```python
from build123d import *

# Parameters (mm, degrees)
EXTRUDE_THIN1_DEPTH  = 100
SKETCH2_R            = 5
CUT_EXTRUDE1_DEPTH   = 10
LPATTERN1_COUNT      = 2
LPATTERN1_PITCH      = 70
SKETCH3_R            = 5
CUT_EXTRUDE2_DEPTH   = 10
LPATTERN2_COUNT      = 3
LPATTERN2_PITCH      = 260
LPATTERN2_COUNT_DIR2 = 2
LPATTERN2_PITCH_DIR2 = 70
SKETCH4_R            = 5
CUT_EXTRUDE3_DEPTH   = 10
LPATTERN3_COUNT      = 2
LPATTERN3_PITCH      = 70


with BuildPart() as part:
    # Sketch1 → Extrude-Thin1 (new body)
    with BuildSketch(Plane.XY):
        with BuildLine():
            Line((0, 0), (0, 126.921326068))
            ThreePointArc((0, 126.921326068), (6.221950993, 145.213520727), (22.306959029, 155.918172804))
            Line((22.306959029, 155.918172804), (735, 345))
            Line((735, 345), (736.282173495, 340.167192211))
            Line((736.282173495, 340.167192211), (23.589132524, 151.085365014))
            ThreePointArc((23.589132524, 151.085365014), (10.184959161, 142.164821617), (5, 126.921326068))
            Line((5, 126.921326068), (5, 0))
            Line((5, 0), (0, 0))
        make_face()
    extrude(amount=EXTRUDE_THIN1_DEPTH)

    # Sketch2 → Cut-Extrude1 (cut)
    with BuildSketch(Plane(origin=(-37.178988327, 140.13618677, 0), x_dir=(0.9665615578617778, 0.25643469902455335, 0), z_dir=(-0.25643469902455335, 0.9665615578617778, 0))):
        with Locations(Location((686.892716192, -15, 0), (0, 0, 180))):
            Circle(SKETCH2_R)
    cut_extrude1 = extrude(amount=-CUT_EXTRUDE1_DEPTH, mode=Mode.SUBTRACT)

    # LPattern1: Cut-Extrude1 ×2
    with Locations(*[(0, 0, i * LPATTERN1_PITCH) for i in range(1, LPATTERN1_COUNT)]):
        add(cut_extrude1, mode=Mode.SUBTRACT)

    # Sketch3 → Cut-Extrude2 (cut)
    with BuildSketch(Plane(origin=(-37.178988327, 140.13618677, 0), x_dir=(0.9665615578617778, 0.25643469902455335, 0), z_dir=(-0.25643469902455335, 0.9665615578617778, 0))):
        with Locations(Location((612.892716192, -15, 0), (0, 0, 180))):
            Circle(SKETCH3_R)
    cut_extrude2 = extrude(amount=-CUT_EXTRUDE2_DEPTH, mode=Mode.SUBTRACT)

    # LPattern2: Cut-Extrude2 3 × 2
    with Locations(*[Vector(-0.9665615578617778, -0.25643469902455335, 0) * (i * LPATTERN2_PITCH) + Vector(0, 0, 1) * (j * LPATTERN2_PITCH_DIR2) for i in range(LPATTERN2_COUNT) for j in range(LPATTERN2_COUNT_DIR2) if (i, j) != (0, 0)]):
        add(cut_extrude2, mode=Mode.SUBTRACT)

    # Sketch4 → Cut-Extrude3 (cut)
    with BuildSketch(Plane.ZY):
        with Locations((85, 20)):
            Circle(SKETCH4_R)
    cut_extrude3 = extrude(amount=-CUT_EXTRUDE3_DEPTH, mode=Mode.SUBTRACT)

    # LPattern3: Cut-Extrude3 ×2
    with Locations(*[(0, 0, -i * LPATTERN3_PITCH) for i in range(1, LPATTERN3_COUNT)]):
        add(cut_extrude3, mode=Mode.SUBTRACT)


solid = part.part
```
Design review of the part built by this model. Coordinates are the model's own, in mm. A direction names the side the tool comes from. Give positions to 0.01 mm unless a question says otherwise; leave off trailing zeros. Write each loop counter-clockwise with the first axis right and the second up, starting at its lowest first coordinate (ties: lowest second). Pieces come first, ordered by that corner, then holes.
(1) Add section C-C (y = 70). Give the boundary of the cut face in (x, z), and give its area (3 significant figures).
Checked values:
outline: (0, 0) - (5, 0) - (5, 100) - (0, 100) - close
area: 500 mm2
(2) Wall thickness on line 1 along X through (y, z) = (114, 18); line 2 along Y through (x, z) = (3, 15); line 3 along Y through (x, z) = (263, 15): over which ranges is each line inside the solid? List them lowest first.
Checked values:
line 1: x = 0 to 5
line 2: y = 0 to 15, 25 to 140
line 3: y = 214.6 to 219.78
(3) Mouldability with a two-part tool opening along Z and no side actions: class faces 1 (the face through (343, 237, 100)), 2 (the face through (384.92, 246.95, 49.3)), 3 (the face through (343, 237, 0)) as +Z half, -Z half, draft (parallel to the pull), parting line (faces both ways), or undercut.
Checked values:
face 1: +Z half
face 2: draft
face 3: -Z half
(4) Add section B-B (x = 438.5). Give the boundary of the cut face in (y, z).
Checked values:
outline: (261.16, 0) - (266.34, 0) - (266.34, 100) - (261.16, 100) - close
(5) Clearance check with flat-ended pins moving along their axes: pin 1 Ø2 at (x, z) = (456, 73) entering from +Y; pin 2 Ø1 at (x, z) = (645, 31) entering from +Y; pin 3 Ø13 at (y, z) = (20, 15) entering from +X. State where each tip first meets the part, or that it passes through.
Checked values:
pin 1: stops at y = 271.24
pin 2: stops at y = 321.26
pin 3: stops at x = 5
(6) Add section A-A (z = 45). Give the boundary of the cut face in (x, y).
Checked values:
outline: (0, 0) - (5, 0) - (5, 126.92) arc R25 cw to (23.59, 151.09) - (736.28, 340.17) - (735, 345) - (22.31, 155.92) arc R30 ccw to (0, 126.92) - close
(7) Tool access review of faces 4 (the face through (5, 64, 49)), 5 (the face through (6.055, 144.994, 49.3)): name each direction out of +Z, -Z, +X, -X, +Y, -Y from which nothing blocks a thin tool from reaching the whole face with its end or side.
Checked values:
face 4: +Z, -Z, +X, -Y
face 5: +Z, -Z, -X, +Y
